from build123d import *

# Parameters (mm, degrees)
SKETCH1_R                  = 215
BOSS_EXTRUDE1_DEPTH        = 40
F_16_0_16_DIAMETER_HOLE1_D = 16
G1_2_TAPPED_HOLE1_D        = 19


with BuildPart() as part:
    # Sketch1 → Boss-Extrude1 (new body)
    with BuildSketch(Plane(origin=(0, 0, 0), x_dir=(1, 0, 0), z_dir=(0, 1, 0))):
        with Locations(Location((0, 0, 0), (0, 0, 270))):
            Circle(SKETCH1_R)
    extrude(amount=BOSS_EXTRUDE1_DEPTH)

    # Ø16.0 (16) Diameter Hole1 (through all)
    with Locations(Plane(origin=(0, 40, 0), x_dir=(1, 0, 0), z_dir=(0, 1, 0))):
        with Locations((200, 0), (190.211303259, -61.803398875), (161.803398875, -117.557050458), (117.557050458, -161.803398875), (61.803398875, -190.211303259), (0, -200), (-61.803398875, -190.211303259), (-117.557050458, -161.803398875), (-161.803398875, -117.557050458), (-190.211303259, -61.803398875), (-200, 0), (-190.211303259, 61.803398875), (-161.803398875, 117.557050458), (-117.557050458, 161.803398875), (-61.803398875, 190.211303259), (0, 200), (61.803398875, 190.211303259), (117.557050458, 161.803398875), (161.803398875, 117.557050458), (190.211303259, 61.803398875)):
            Hole(F_16_0_16_DIAMETER_HOLE1_D / 2)

    # G1/2 Tapped Hole1 (through all)
    with Locations(Plane(origin=(0, 40, 0), x_dir=(1, 0, 0), z_dir=(0, 1, 0))):
        with Locations((-60, 0), (60, 0)):
            Hole(G1_2_TAPPED_HOLE1_D / 2)


solid = part.part
Part model, mm, in its own coordinate system. Coordinates: 2 decimals unless noted, no trailing zeros. Order: outer loops, then holes, each group sorted by start corner. A loop starts at its lowest first (then second) coordinate and runs counter-clockwise, first axis right, second up.
(1) Slice it at B-B, the plane y = 15.5. State how many separate pieces and enclosed holes the cut face has, and give its area (3 significant figures).
Check sheet entries:
separate pieces: 1
enclosed holes: 22
area: 141,000 mm2
(2) Slice it at D-D, the plane z = 103. Write the cut outline in (x, y).
Check sheet entries:
outline: (-188.72, 0) - (188.72, 0) - (188.72, 40) - (-188.72, 40) - close
(3) Pin check, flat tips, straight feed: pin 1 Ø9.5 at (x, z) = (0, -200) entering from -Y; pin 2 Ø4 at (x, y) = (28.5, 8) entering from -Z; pin 3 Ø5 at (y, z) = (14, 68.5) entering from +X; pin 4 Ø5 at (x, y) = (158.5, 24) entering from -Z. Stop position of each tip, or through.
Check sheet entries:
pin 1: passes through
pin 2: stops at z = -213.36
pin 3: stops at x = 204.62
pin 4: stops at z = -147.95
(4) Probe L1, parallel to Z at x = 158.5, y = 29; L2, parallel to X at y = 21, z = 193; L3, parallel to X at y = 12, z = 183.5. List the from-to ranges inside material, lowest first.
Check sheet entries:
L1: z = -145.27 to -124.84, -110.27 to 110.27, 124.84 to 145.27
L2: x = -94.74 to -69.3, -54.31 to -3.87, 3.87 to 54.31, 69.3 to 94.74
L3: x = -112.04 to -66.16, -57.45 to 57.45, 66.16 to 112.04
(5) Slice it at A-A, the plane x = 0. Write the cut outline in (y, z).
Check sheet entries:
outline: (0, -215) - (40, -215) - (40, -208) - (0, -208) - close; (0, -192) - (40, -192) - (40, 192) - (0, 192) - close; (0, 208) - (40, 208) - (40, 215) - (0, 215) - close
(6) Slice it at C-C, the plane x = 60. Write the cut outline in (y, z).
Check sheet entries:
outline: (0, -206.46) - (40, -206.46) - (40, -198.01) - (0, -198.01) - close; (0, -182.42) - (40, -182.42) - (40, -9.5) - (0, -9.5) - close; (0, 9.5) - (40, 9.5) - (40, 182.42) - (0, 182.42) - close; (0, 198.01) - (40, 198.01) - (40, 206.46) - (0, 206.46) - close
(7) Pull direction Z, two halves, no side cores. Call faces 1 (the face through (3, 0, -3)), 2 (the face through (-121.86, 19.72, -168.55)): pulls with the +Z half, pulls with the -Z half, needs draft (parallel to the pull), parting line crosses it, or undercut.
Check sheet entries:
face 1: needs draft
face 2: undercut
